Part model, mm, in its own coordinate system. Give positions to 0.01 mm unless a question says otherwise; leave off trailing zeros. Write each loop counter-clockwise with the first axis right and the second up, starting at its lowest first coordinate (ties: lowest second). Pieces come first, ordered by that corner, then holes. Notation, with made-up numbers: M -38.5,28.5 L 15.5,28.5 A26 ccw 15.5,49.5 Z; hole C 67,38.25 d3. An arc over 180 degrees is marked long. Use a Markdown table: item, result. Add a question column.
from build123d import *

# Parameters (mm, degrees)
BOSS_EXTRUDE1_DEPTH = 30
M10_TAPPED_HOLE1_D  = 8.5


with BuildPart() as part:
    # Sketch1 → Boss-Extrude1 (new body)
    with BuildSketch(Plane.XY):
        with BuildLine():
            Line((-107, 0), (-107, 23.5))
            Line((-107, 23.5), (107, 23.5))
            Line((107, 23.5), (107, 0))
            Line((107, 0), (105.431676725, 0))
            ThreePointArc((105.431676725, 0), (104.420376931, 0.392176581), (103.937887932, 1.363636364))
            ThreePointArc((103.937887932, 1.363636364), (88.317474901, 14.984463937), (74, 0))
            ThreePointArc((74, 0), (72.5, -1.5), (71, 0))
            ThreePointArc((71, 0), (56, 15), (41, 0))
            ThreePointArc((41, 0), (39.5, -1.5), (38, 0))
            ThreePointArc((38, 0), (23.682525099, 14.984463937), (8.062112068, 1.363636364))
            ThreePointArc((8.062112068, 1.363636364), (7.579623069, 0.392176581), (6.568323275, 0))
            Line((6.568323275, 0), (-6.568323275, 0))
            ThreePointArc((-6.568323275, 0), (-7.579623069, 0.392176581), (-8.062112068, 1.363636364))
            ThreePointArc((-8.062112068, 1.363636364), (-23.682525099, 14.984463937), (-38, 0))
            ThreePointArc((-38, 0), (-39.5, -1.5), (-41, 0))
            ThreePointArc((-41, 0), (-56, 15), (-71, 0))
            ThreePointArc((-71, 0), (-72.5, -1.5), (-74, 0))
            ThreePointArc((-74, 0), (-88.317474901, 14.984463937), (-103.937887932, 1.363636364))
            ThreePointArc((-103.937887932, 1.363636364), (-104.420376931, 0.392176581), (-105.431676725, 0))
            Line((-105.431676725, 0), (-107, 0))
        make_face()
    extrude(amount=BOSS_EXTRUDE1_DEPTH)

    # M10 Tapped Hole1 (through all)
    with Locations(Plane(origin=(0, 23.5, 0), x_dir=(-1, 0, 0), z_dir=(0, 1, 0))):
        with Locations((0, 15)):
            Hole(M10_TAPPED_HOLE1_D / 2)


solid = part.part
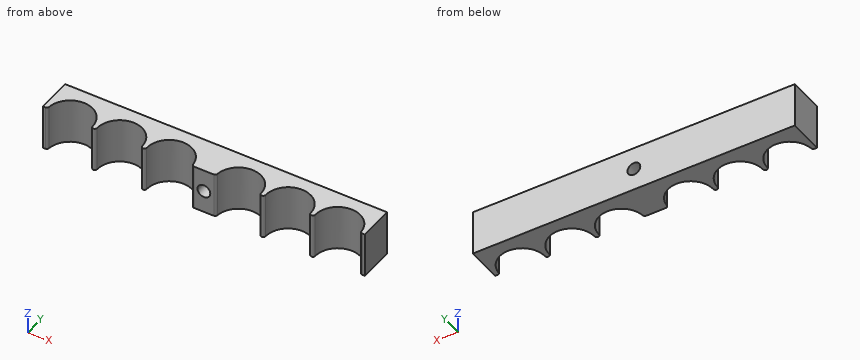
1. Cut at B-B (x = 0). Write the cut outline in (y, z), then the cut area to 3 significant figures.
2. Flat gauge pins, fed straight in: pin 1 (1.3 mm diameter, centred on x = -106.5, z = 8, fed in from -Y); pin 2 (6 mm diameter, centred on x = 63, z = 8.5, fed in from -Y). Where does each tip first touch, or does it go through?
3. Drill centre lines: probe 1 along Z at (x, y) = (0, 11); probe 2 along Y at (x, z) = (6.5, 17); probe 3 along Y at (x, z) = (-12.5, 28.75). Where is each one in solid material? Low to high. Write a range as [from, to].
4. Cut at A-A (z = 15). Write the cut outline in (x, y), then the cut area to 3 significant figures.
5. Cut at C-C (y = 4.5). Give the number of separate pieces and of enclosed holes in the cut face, then the cut area to 3 significant figures.
6. Cut at D-D (x = -56). Write the cut outline in (y, z), then the cut area to 3 significant figures.
A:
| question | item | result |
|---|---|---|
| 1 | outline | M 0,0 L 23.5,0 L 23.5,10.75 L 0,10.75 Z; M 0,19.25 L 23.5,19.25 L 23.5,30 L 0,30 Z |
| 1 | area | 505 mm² |
| 2 | pin 1 | stops at y = 0 |
| 2 | pin 2 | stops at y = 11.18 |
| 3 | probe 1 | z = [0, 10.75], [19.25, 30] |
| 3 | probe 2 | y = [0, 23.5] |
| 3 | probe 3 | y = [10.71, 23.5] |
| 4 | outline | M -107,0 L -105.43,0 A1.5 ccw -103.94,1.36 A15 cw -74,0 A1.5 ccw -71,0 A15 cw -41,0 A1.5 ccw -38,0 A15 cw -8.06,1.36 A1.5 ccw -6.57,0 L -4.25,0 L -4.25,23.5 L -107,23.5 Z; M 4.25,0 L 6.57,0 A1.5 ccw 8.06,1.36 A15 cw 38,0 A1.5 ccw 41,0 A15 cw 71,0 A1.5 ccw 74,0 A15 cw 103.94,1.36 A1.5 ccw 105.43,0 L 107,0 L 107,23.5 L 4.25,23.5 Z |
| 4 | area | 2,720 mm² |
| 5 | separate pieces | 7 |
| 5 | enclosed holes | 1 |
| 5 | area | 1,210 mm² |
| 6 | outline | M 15,0 L 23.5,0 L 23.5,30 L 15,30 Z |
| 6 | area | 255 mm² |
